Geometry check sheet. Reference: the model listing, model coordinates, mm. Face numbers are marked on the shaded views. A direction names the side the tool comes from. Give positions to 0.01 mm unless a question says otherwise; leave off trailing zeros. Write each loop counter-clockwise with the first axis right and the second up, starting at its lowest first coordinate (ties: lowest second). Pieces come first, ordered by that corner, then holes. Notation, with made-up numbers: (54.25, 14.25) -> (98.25, 14.25) arc R23 ccw to (98.25, 37.25) -> close; hole circle Ø4 at (19.25, 58.25). An arc over 180 degrees is marked (long way). One line per item, written item: value.
from build123d import *

# Parameters (mm, degrees)
SKETCH_1_W                = 30
SKETCH_1_H                = 30
EXTRUDE_1_DEPTH           = 100
HOLE_WIZARD_1_D           = 11
HOLE_WIZARD_1_CBORE_D     = 18
HOLE_WIZARD_1_CBORE_DEPTH = 11
HOLE_WIZARD_M10_1_D       = 8.5


with BuildPart() as part:
    # 草图1 → 凸台-拉伸1 (new body)
    with BuildSketch(Plane(origin=(0, 0, 0), x_dir=(1, 0, 0), z_dir=(0, 1, 0))):
        Rectangle(SKETCH_1_W, SKETCH_1_H)
    extrude(amount=EXTRUDE_1_DEPTH)

    # 打孔尺寸(%根据)内六角圆柱头螺钉的类型1 (through all)
    with Locations(Plane(origin=(0, 0, -15), x_dir=(-1, 0, 0), z_dir=(0, 0, -1))):
        with Locations((0, 15), (0, 85)):
            CounterBoreHole(HOLE_WIZARD_1_D / 2, HOLE_WIZARD_1_CBORE_D / 2, HOLE_WIZARD_1_CBORE_DEPTH)

    # M10 螺纹孔1 (through all)
    with Locations(Plane.ZY.offset(15)):
        with Locations((5, 50)):
            Hole(HOLE_WIZARD_M10_1_D / 2)


solid = part.part
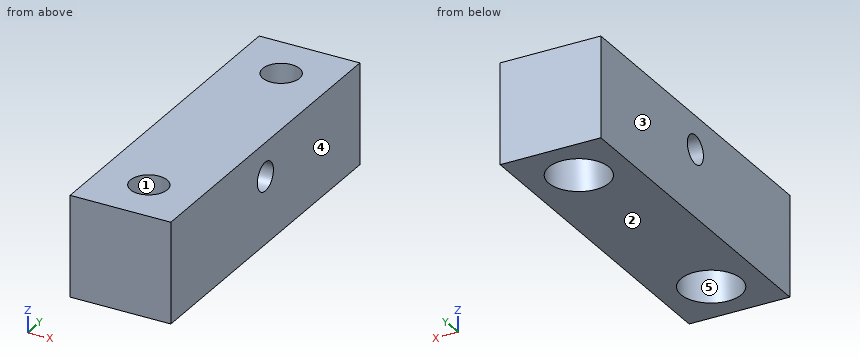
1) Sectioned sample at C-C on y = 85. Record the cut outline in (x, z), plus the area to 3 significant figures.
Verdict:
outline: (-15, -15) -> (-9, -15) -> (-9, -4) -> (-5.5, -4) -> (-5.5, 15) -> (-15, 15) -> close; (5.5, -4) -> (9, -4) -> (9, -15) -> (15, -15) -> (15, 15) -> (5.5, 15) -> close
area: 493 mm^2
2) Depth check by flat-ended pin: pin 1 Ø12 at (x, y) = (-6, 78.5) entering from -Z; pin 2 Ø9 at (x, y) = (1, 83.5) entering from -Z. Enter the tip coordinate at first touch or a pass-through.
Verdict:
pin 1: z = -15
pin 2: z = -4
3) Sectioned sample at B-B on x = 0. Record the cut outline in (y, z), plus the area to 3 significant figures.
Verdict:
outline: (0, -15) -> (6, -15) -> (6, -4) -> (9.5, -4) -> (9.5, 15) -> (0, 15) -> close; (20.5, -4) -> (24, -4) -> (24, -15) -> (76, -15) -> (76, -4) -> (79.5, -4) -> (79.5, 15) -> (20.5, 15) -> close; (90.5, -4) -> (94, -4) -> (94, -15) -> (100, -15) -> (100, 15) -> (90.5, 15) -> close; hole circle Ø8.5 at (50, 5)
area: 2,130 mm^2
4) Scan lines: probe 1 along Y at (x, z) = (0, -8.25); probe 2 along Y at (x, z) = (0, 4.5); probe 3 along Y at (x, z) = (5.75, -12.75). Record each from-to range of solid material in increasing order.
Verdict:
probe 1: 0 to 6, 24 to 76, 94 to 100
probe 2: 0 to 9.5, 20.5 to 45.78, 54.22 to 79.5, 90.5 to 100
probe 3: 0 to 8.08, 21.92 to 78.08, 91.92 to 100
5) Mould release check, pull along X, two halves, no side actions. Record for the marked faces 1, 2 and 3: released by +X, released by -X, zero draft, split by the parting line, or undercut.
Verdict:
face 1: undercut
face 2: zero draft
face 3: released by -X
6) Sectioned sample at D-D on z = -5.25. Record the cut outline in (x, y).
Verdict:
outline: (-15, 0) -> (15, 0) -> (15, 100) -> (-15, 100) -> close; hole circle Ø18 at (0, 15); hole circle Ø18 at (0, 85)
7) Sectioned sample at A-A on z = 5. Record the cut outline in (x, y).
Verdict:
outline: (-15, 0) -> (15, 0) -> (15, 45.75) -> (-15, 45.75) -> close; (-15, 54.25) -> (15, 54.25) -> (15, 100) -> (-15, 100) -> close; hole circle Ø11 at (0, 15); hole circle Ø11 at (0, 85)
8) Tool access check on the marked faces 4 and 5. Record the directions out of +Z, -Z, +X, -X, +Y, -Y that give a thin tool (end or side, any length) a straight path to the whole face; none if there is none.
Verdict:
face 4: +Z, -Z, +X, +Y, -Y
face 5: -Z
